Could you check a few things on this drawing? It's one solid part, dimensions in mm from its lowest x, y, z. Give positions to 0.01 mm unless a question says otherwise; leave off trailing zeros. Write each loop counter-clockwise with the first axis right and the second up, starting at its lowest first coordinate (ties: lowest second). Pieces come first, ordered by that corner, then holes. Notation, with made-up numbers: (-21, 64.5) - (-11, 64.5) arc R18 cw to (-11, 99.5) - close; hole circle Ø5 at (71, 1.5). An arc over 180 degrees is marked (long way). One line per item, written item: value. Start each with the question number.
1) Imagine slicing it at A-A on z = 6.75. Write out the boundary of the cut face in (x, y).
2) Imagine slicing it at B-B on y = 18. Write out the boundary of the cut face in (x, z) (3 decimals), plus the area to 3 significant figures.
3) Please list where these lines run through material, in increasing order: L1, parallel to Y at x = 226, z = 7.75; L2, parallel to Y at x = 34.5, z = 7.25; L3, parallel to X at y = 22, z = 8 (3 decimals). Write a range as [from, to].
4) I'm going to push flat-ended pins straight in: P1, Ø1, axis at y = 27.5, z = 2, coming from the -X side; P2, Ø1, axis at y = 15, z = 5.5, coming from the -X side. Where does each tip first touch, or does it pass through?
5) Imagine slicing it at C-C on x = 34. Write out the boundary of the cut face in (y, z), plus the area to 3 significant figures.
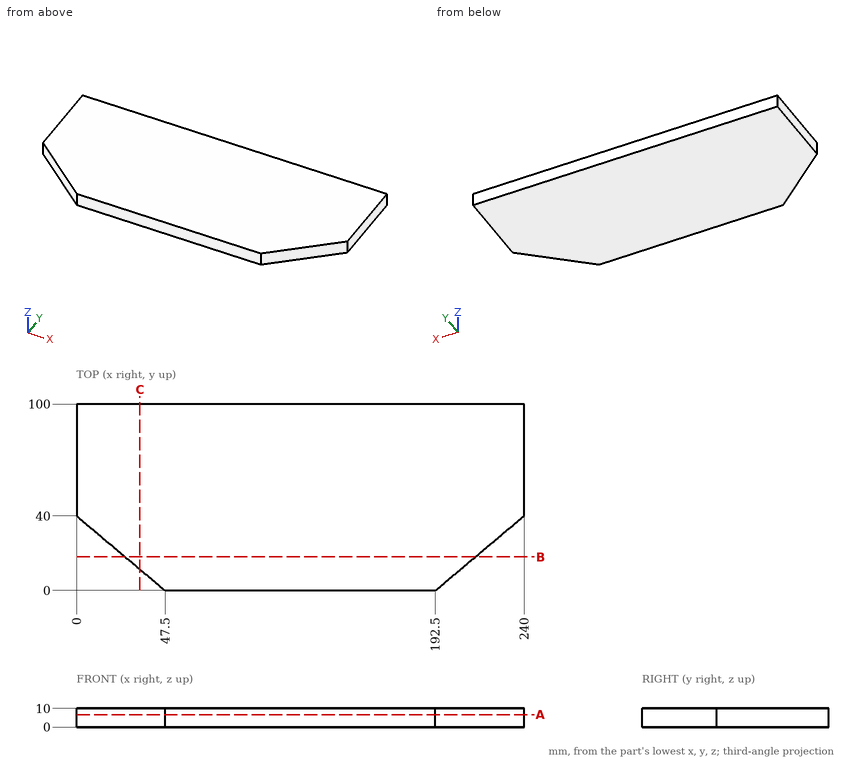
Numbers:
1. outline: (0, 40) - (47.5, 0) - (192.5, 0) - (240, 40) - (240, 100) - (0, 100) - close
2. outline: (26.125, 0) - (213.875, 0) - (213.875, 10) - (26.125, 10) - close
2. area: 1,880 mm^2
3. L1: [28.21, 100]
3. L2: [10.95, 100]
3. L3: [21.375, 218.625]
4. P1: x = 14.25
4. P2: x = 29.09
5. outline: (11.37, 0) - (100, 0) - (100, 10) - (11.37, 10) - close
5. area: 886 mm^2
